For this review, use the dimensioned drawing (mm, ordinates from the lowest corner) and the shaded views. Give positions to 0.01 mm unless a question says otherwise; leave off trailing zeros. Write each loop counter-clockwise with the first axis right and the second up, starting at its lowest first coordinate (ties: lowest second). Pieces come first, ordered by that corner, then holes. Notation, with made-up numbers: (40.25, -26.5) -> (96.25, -26.5) arc R25 ccw to (96.25, -7.5) -> close; hole circle Ø10 at (73.5, -17). An arc over 180 degrees is marked (long way). Return JSON: item names as keys, results as strings.
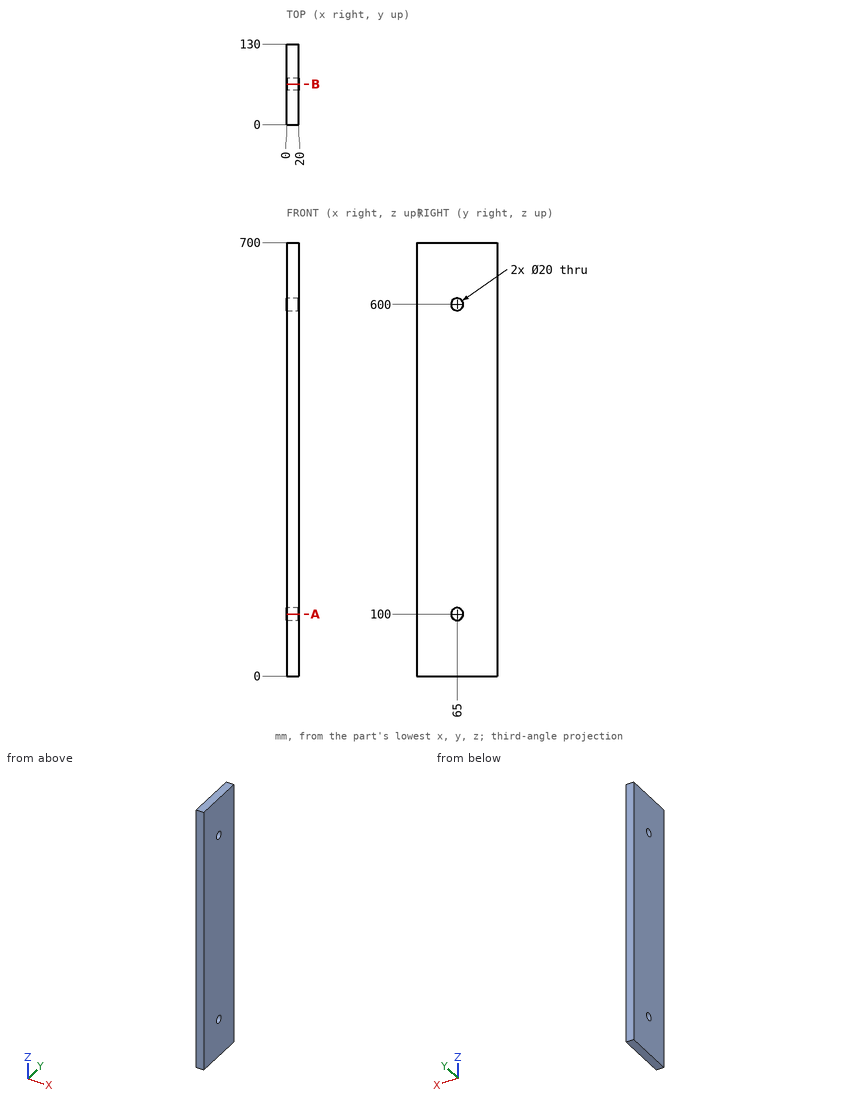
1. Add section B-B, the plane y = 65. State the section outline as (x, z) points.
Results found:
{"outline": "(0, 0) -> (20, 0) -> (20, 90) -> (0, 90) -> close; (0, 110) -> (20, 110) -> (20, 590) -> (0, 590) -> close; (0, 610) -> (20, 610) -> (20, 700) -> (0, 700) -> close"}
2. Add section A-A, the plane z = 100. State the section outline as (x, y) points, plus the area to 3 significant figures.
Results found:
{"outline": "(0, 0) -> (20, 0) -> (20, 55) -> (0, 55) -> close; (0, 75) -> (20, 75) -> (20, 130) -> (0, 130) -> close", "area": "2,200 mm²"}
3. To check wall thickness, follow probe 1 along Y at (x, z) = (11, 100); probe 2 along Z at (x, y) = (11.5, 63); probe 3 along Z at (x, y) = (9.5, 58). State the ranges of each line that lie inside material, in increasing order.
Results found:
{"probe 1": "y = 0 to 55, 75 to 130", "probe 2": "z = 0 to 90.2, 109.8 to 590.2, 609.8 to 700", "probe 3": "z = 0 to 92.86, 107.14 to 592.86, 607.14 to 700"}
